from build123d import *

# Parameters (mm, degrees)
BOSS_EXTRUDE1_DEPTH     = 20
SKETCH2_R               = 2
CUT_EXTRUDE1_DEPTH      = 69.190908485
CUT_EXTRUDE2_DEPTH      = 69.738635424
CUT_EXTRUDE2_DEPTH_BACK = 69.738635424
SKETCH3_W               = 70
SKETCH3_H               = 12
CUT_EXTRUDE3_DEPTH      = 69.190908485
CUT_EXTRUDE3_DEPTH_BACK = 69.190908485
SKETCH4_R               = 2
SKETCH5_R               = 2.5
BOSS_EXTRUDE2_DEPTH     = 16
SKETCH6_R               = 1.5
BOSS_EXTRUDE3_DEPTH     = 16
BOSS_EXTRUDE4_START     = -16
BOSS_EXTRUDE4_DEPTH     = 6
CUT_EXTRUDE4_DEPTH      = 69.667677986
CUT_EXTRUDE4_DEPTH_BACK = 69.667677986
SKETCH8_R               = 0.52328701
SKETCH9_W               = 3.261997226
SKETCH9_H               = 3.598658034
BOSS_EXTRUDE5_DEPTH     = 4
SKETCH10_W              = 3.703262865
SKETCH10_H              = 2.596843015
BOSS_EXTRUDE6_DEPTH     = 6


with BuildPart() as part:
    # Sketch1 → Boss-Extrude1 (new body)
    with BuildSketch(Plane(origin=(0, 0, 0), x_dir=(1, 0, 0), z_dir=(0, 1, 0))):
        with BuildLine():
            Line((-5, 0), (-5, -60))
            ThreePointArc((-5, -60), (0, -65), (5, -60))
            Line((5, -60), (5, 0))
            ThreePointArc((5, 0), (0, 5), (-5, 0))
        make_face()
    extrude(amount=BOSS_EXTRUDE1_DEPTH)

    # Sketch2 → Cut-Extrude1 (cut, through all)
    with BuildSketch(Plane(origin=(0, 20, 0), x_dir=(1, 0, 0), z_dir=(0, 1, 0))):
        with Locations(Location((0, 0, 0), (0, 0, 270))):
            Circle(SKETCH2_R)
        with Locations(Location((0, -16.5, 0), (0, 0, 270))):
            Circle(SKETCH2_R)
    extrude(amount=-CUT_EXTRUDE1_DEPTH, mode=Mode.SUBTRACT)

    # Sketch3 → Cut-Extrude2 (cut, two sides: drawn at the far end of the back side and taken through both)
    with BuildSketch(Plane(origin=(5, 0, 0), x_dir=(0, 0, -1), z_dir=(1, 0, 0)).offset(-CUT_EXTRUDE2_DEPTH_BACK)):
        with Locations((-30, 10)):
            Rectangle(SKETCH3_W, SKETCH3_H)
    extrude(amount=CUT_EXTRUDE2_DEPTH + CUT_EXTRUDE2_DEPTH_BACK, mode=Mode.SUBTRACT)


with BuildPart() as cut_extrude2_piece_1:
    # of the separate pieces the step leaves, piece 1, a body of its own (cut_extrude2_pieces)
    add(part.part.solids().sort_by_distance((5, 16, 60))[0])


with BuildPart() as cut_extrude2_piece_2:
    # of the separate pieces the step leaves, piece 2, a body of its own (cut_extrude2_pieces)
    add(part.part.solids().sort_by_distance((5, 0, 60))[0])


with BuildPart() as cut_extrude3_tool:
    # Sketch4 → Cut-Extrude3 (new, two sides: drawn at the far end of the back side and taken through both)
    with BuildSketch(Plane(origin=(0, 20, 0), x_dir=(1, 0, 0), z_dir=(0, 1, 0)).offset(-CUT_EXTRUDE3_DEPTH_BACK)):
        with Locations(Location((0, -60, 0), (0, 0, 270))):
            Circle(SKETCH4_R)
    extrude(amount=CUT_EXTRUDE3_DEPTH + CUT_EXTRUDE3_DEPTH_BACK)


with BuildPart() as cut_extrude2_piece_1_1:
    add(cut_extrude2_piece_1.part)

    # Cut-Extrude3: cut by cut_extrude3_tool
    add(cut_extrude3_tool.part, mode=Mode.SUBTRACT)



with BuildPart() as cut_extrude2_piece_2_1:
    add(cut_extrude2_piece_2.part)

    # Cut-Extrude3: cut by cut_extrude3_tool
    add(cut_extrude3_tool.part, mode=Mode.SUBTRACT)


with BuildPart() as cut_extrude2_piece_1_2:
    add(cut_extrude2_piece_1_1.part)

    add(cut_extrude2_piece_2_1.part)  # Boss-Extrude2 merges Cut-Extrude2 piece 2
    # Sketch5 → Boss-Extrude2 (add)
    with BuildSketch(Plane(origin=(0, 20, 0), x_dir=(1, 0, 0), z_dir=(0, 1, 0))):
        with Locations(Location((0, -34.552446897, 0), (0, 0, 270))):
            Circle(SKETCH5_R)
    extrude(amount=-BOSS_EXTRUDE2_DEPTH)

    # Sketch6 → Boss-Extrude3 (add)
    with BuildSketch(Plane(origin=(0, 20, 0), x_dir=(1, 0, 0), z_dir=(0, 1, 0))):
        with Locations(Location((-2, -50, 0), (0, 0, 270))):
            Circle(SKETCH6_R)
    extrude(amount=-BOSS_EXTRUDE3_DEPTH)

    # Sketch7 → Boss-Extrude4 (add)
    with BuildSketch(Plane(origin=(0, 20, 0), x_dir=(1, 0, 0), z_dir=(0, 1, 0)).offset(BOSS_EXTRUDE4_START)):
        Polygon((4.5, -38), (-4, -38), (-4, -48), (4.5, -48), (4.5, -44), align=None)
    extrude(amount=BOSS_EXTRUDE4_DEPTH)

    # Sketch8 → Cut-Extrude4 (cut, two sides: drawn at the far end of the back side and taken through both)
    with BuildSketch(Plane(origin=(4.5, 0, 0), x_dir=(0, 0, -1), z_dir=(1, 0, 0)).offset(-CUT_EXTRUDE4_DEPTH_BACK)):
        with Locations((-39.788503734, 6.691891051)):
            Circle(SKETCH8_R)
        with Locations((-46.515921266, 6.691891051)):
            Circle(SKETCH8_R)
        with Locations((-43.19958868, 8.823819142)):
            Circle(SKETCH8_R)
    extrude(amount=CUT_EXTRUDE4_DEPTH + CUT_EXTRUDE4_DEPTH_BACK, mode=Mode.SUBTRACT)

    # Sketch9 → Boss-Extrude5 (add)
    with BuildSketch(Plane(origin=(0, 10, 0), x_dir=(1, 0, 0), z_dir=(0, 1, 0))):
        with Locations((0.25, -43)):
            Rectangle(SKETCH9_W, SKETCH9_H)
    extrude(amount=BOSS_EXTRUDE5_DEPTH)

    # Sketch10 → Boss-Extrude6 (add)
    with BuildSketch(Plane(origin=(0, 10, 0), x_dir=(1, 0, 0), z_dir=(0, 1, 0))):
        with Locations((0.168234256, -39.807752572)):
            Rectangle(SKETCH10_W, SKETCH10_H)
        with Locations((0.168234256, -46.192247429)):
            Rectangle(SKETCH10_W, SKETCH10_H)
    extrude(amount=BOSS_EXTRUDE6_DEPTH)


solid = cut_extrude2_piece_1_2.part
Build history of the part. All positions in model axes, mm. A direction names the side the tool comes from. Coordinates: 2 decimals unless noted, no trailing zeros. Write each loop counter-clockwise with the first axis right and the second up, starting at its lowest first coordinate (ties: lowest second). Pieces come first, ordered by that corner, then holes.
(1) Cut at B-B on y = 18.5. List the corners of the cut face in (x, z).
(2) 3-axis set-ups, long thin cutter, end or side, ignore diameter. For faces 1 (the flat face through (-1.683, 13, 46)), 2 (the flat face through (4.5, 7, 43)), 3 (the flat face through (0, 7, 48)), 4 (the cylindrical face through (-0.96, 10.08, 36.86)): which of +Z, -Z, +X, -X, +Y, -Y reach the whole face in a straight line?
(3) Mould opens along Z. For faces 5 (the flat face through (0, 13, 38.509)), 6 (the flat face through (-5, 2, 30)), 7 (the cylindrical face through (0, 2, 65)) say: pulls with the +Z half, pulls with the -Z half, needs draft (parallel to the pull), parting line crosses it, or undercut.
(4) Cut at A-A on z = 53. List the corners of the cut face in (x, y).
(5) Pin check, flat tips, straight feed: pin 1 Ø6 at (x, y) = (-1.5, 11.5) entering from +Z; pin 2 Ø3 at (y, z) = (13, 39.5) entering from +X; pin 3 Ø3 at (y, z) = (12, 39) entering from -X. Stop position of each tip, or through.
(6) Drill centre lines: line 1 (Y direction, x = -3.75, z = 35); line 2 (Z direction, x = 1.25, y = 9.25); line 3 (X direction, y = 2.65, z = 16.5). Where is each one in solid material? Low to high.
Working result:
1. outline: (-5, 0) arc R5 ccw to (5, 0) - (5, 60) arc R5 ccw to (-5, 60) - close; hole circle Ø4 at (0, 0); hole circle Ø4 at (0, 16.5); hole circle Ø4 at (0, 60)
2. face 1: -X
2. face 2: +Z, -Z, +X
2. face 3: +X, -X
2. face 4: none
3. face 5: undercut
3. face 6: needs draft
3. face 7: pulls with the +Z half
4. outline: (-5, 0) - (5, 0) - (5, 4) - (-5, 4) - close; (-5, 16) - (5, 16) - (5, 20) - (-5, 20) - close
5. pin 1: stops at z = 51.5
5. pin 2: stops at x = 2.02
5. pin 3: stops at x = -1.68
6. line 1: y = 0 to 4, 16 to 20
6. line 2: z = 32.39 to 36.72, 38 to 42.9, 43.5 to 48
6. line 3: x = -5 to -2, 2 to 5
